Can you work these out from the model? Positions are in its coordinate system, mm. A direction names the side the tool comes from. Give positions to 0.01 mm unless a question says otherwise; leave off trailing zeros. Write each loop counter-clockwise with the first axis right and the second up, starting at its lowest first coordinate (ties: lowest second). Pieces come first, ordered by that corner, then holes. Notation, with made-up numbers: M -31,85.5 L 11,85.5 A35 cw 11,123.5 Z; hole C -39,-0.5 d1. An arc over 180 degrees is marked long. Write each question's results on one line, items separated by ' | '.
from build123d import *

# Parameters (mm, degrees)
SKETCH_1_R      = 75
SKETCH_1_R_2    = 15
EXTRUDE_1_DEPTH = 60


with BuildPart() as part:
    # 草图1 → 凸台-拉伸1 (new body)
    with BuildSketch(Plane.XY):
        Circle(SKETCH_1_R)
        Circle(SKETCH_1_R_2, mode=Mode.SUBTRACT)
    extrude(amount=EXTRUDE_1_DEPTH)

    # 草图2 → 切除-旋转2 (revolve, cut)
    with BuildSketch(Plane(origin=(0, 0, 0), x_dir=(1, 0, 0), z_dir=(0, 1, 0)), mode=Mode.PRIVATE) as cut_revolve_2_sk:
        Polygon((-75, -46.866291189), (-75, -58.022292434), (-64.263367228, -52.307244529), (-64.263367228, -51.572801228), align=None)
        Polygon((-75, -32.38659394), (-75, -43.542595186), (-64.263367228, -37.827547281), (-64.263367228, -37.09310398), align=None)
        Polygon((-75, -17.906896692), (-75, -29.062897938), (-64.263367228, -23.347850033), (-64.263367228, -22.613406731), align=None)
        Polygon((-75, -3.427199444), (-75, -14.583200689), (-64.263367228, -8.868152785), (-64.263367228, -8.133709483), align=None)
    revolve(cut_revolve_2_sk.sketch.rotate(Axis((0, 0, 0), (0, 0, -1)), 180), axis=Axis((0, 0, 0), (0, 0, -1)), mode=Mode.SUBTRACT)


solid = part.part
Item 1: If I drill on line 1 (Y direction, x = 0, z = 23); line 2 (Y direction, x = -3, z = 34); line 3 (X direction, y = 8, z = 52), over which ranges is the centre line in solid material (lowest first)? Write a range as from..to.
Geometry says:
line 1: y = -64.26..-15, 15..64.26 | line 2: y = -71.26..-14.7, 14.7..71.26 | line 3: x = -63.76..-12.69, 12.69..63.76
Item 2: I want a section at A-A, the plane z = 49.5. Please give me the cut outline in (x, y).
Geometry says:
outline: C 0,0 d137.98; hole C 0,0 d30
Item 3: I'm going to push flat-ended pins straight in: pin 1 (8 mm diameter, centred on y = -39.5, z = 42, fed in from +X); pin 2 (4 mm diameter, centred on x = -5, z = 38.5, fed in from -Y); pin 3 (6 mm diameter, centred on y = 26.5, z = 7.5, fed in from -X). Where does each tip first touch, or does it pass through?
Geometry says:
pin 1: stops at x = 65.9 | pin 2: stops at y = -69.11 | pin 3: stops at x = -67.63
Item 4: For faces 1 (the face through (16, 1, 60)), 2 (the face through (61.793, -19.46, 52.585)), which set-ups out of +Z, -Z, +X, -X, +Y, -Y let a thin tool reach every point of the face, with its end or its side?
Geometry says:
face 1: +Z, +X, -X, +Y, -Y | face 2: none
Item 5: Thinking about a two-plate mould opening in X: for faces 3 (the face through (61.793, -19.46, 23.625)), 4 (the face through (-14.985, 0.66, 29.58)), 5 (the face through (16, 1, 0)), which applies, +X half, -X half, draft (parallel to the pull), parting line (faces both ways), or undercut?
Geometry says:
face 3: parting line | face 4: undercut | face 5: draft
